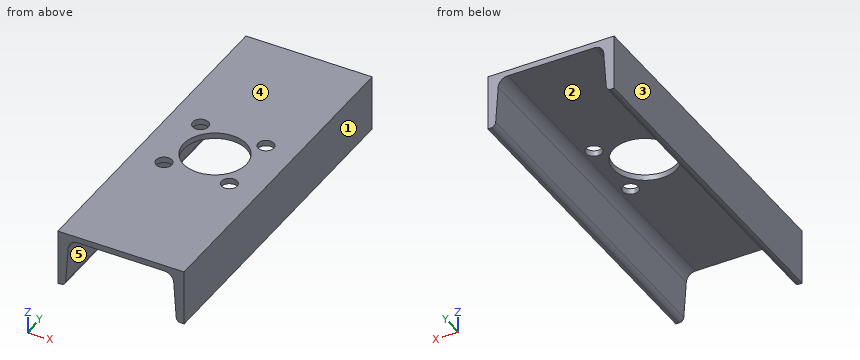
from build123d import *

# Parameters (mm, degrees)
MEMBER_12_1_DEPTH   = 320
SKETCH_5_R          = 30
SKETCH_5_R_2        = 7.5
CUT_EXTRUDE_1_DEPTH = 10


with BuildPart() as part:
    # Sketch1 → Member 12_1 (new body)
    with BuildSketch(Plane.ZX):
        with BuildLine():
            Line((0, 0), (0, -120))
            Line((0, -120), (-53, -120))
            Line((-53, -120), (-53, -117.0157841))
            ThreePointArc((-53, -117.0157841), (-51.788791155, -113.944326346), (-48.807176562, -112.526280502))
            Line((-48.807176562, -112.526280502), (-13.885646876, -110.136912681))
            ThreePointArc((-13.885646876, -110.136912681), (-7.922417689, -107.300820993), (-5.5, -101.157905484))
            Line((-5.5, -101.157905484), (-5.5, -18.842094516))
            ThreePointArc((-5.5, -18.842094516), (-7.922417689, -12.699179007), (-13.885646876, -9.863087319))
            Line((-13.885646876, -9.863087319), (-48.807176562, -7.473719498))
            ThreePointArc((-48.807176562, -7.473719498), (-51.788791155, -6.055673654), (-53, -2.9842159))
            Line((-53, -2.9842159), (-53, 0))
            Line((-53, 0), (0, 0))
        make_face()
    extrude(amount=MEMBER_12_1_DEPTH)

    # 草图5 → 切除-拉伸1 (cut)
    with BuildSketch(Plane.XY):
        with Locations((-60, 160)):
            Circle(SKETCH_5_R)
        with Locations((-91.112698372, 191.112698372)):
            Circle(SKETCH_5_R_2)
        with Locations((-28.887301628, 191.112698372)):
            Circle(SKETCH_5_R_2)
        with Locations((-28.887301628, 128.887301628)):
            Circle(SKETCH_5_R_2)
        with Locations((-91.112698372, 128.887301628)):
            Circle(SKETCH_5_R_2)
    extrude(amount=-CUT_EXTRUDE_1_DEPTH, mode=Mode.SUBTRACT)


solid = part.part
Read the model definition and answer for the solid it produces. Units are mm, in the model's axes. Face numbers are marked on the shaded views. A direction names the side the tool comes from. Round coordinates to 2 decimals unless told otherwise and drop trailing zeros. Write each loop counter-clockwise with the first axis right and the second up, starting at its lowest first coordinate (ties: lowest second). Pieces come first, ordered by that corner, then holes. Notation, with made-up numbers: (-36.75, 7) - (-3.75, 7) arc R12 ccw to (-3.75, 13) - close; hole circle Ø6 at (20.25, -3). An arc over 180 degrees is marked (long way). Use a Markdown table: item, result.
(1) The mould has two halves that part along X. Classify the marked faces 3, 4 and 5: released by +X, released by -X, zero draft, split by the parting line, or undercut.
Reported:
| item | result |
|---|---|
| face 3 | released by -X |
| face 4 | zero draft |
| face 5 | undercut |
(2) Each of these flat-tipped pins is pushed along its axis until it touches: pin 1 Ø17 at (x, y) = (-91.11, 128.89) entering from +Z; pin 2 Ø5 at (x, y) = (-30, 147.5) entering from -Z; pin 3 Ø9 at (x, y) = (-28.89, 191.11) entering from -Z. Where does it stop, or does it pass through?
Reported:
| item | result |
|---|---|
| pin 1 | z = 0 |
| pin 2 | z = -5.5 |
| pin 3 | through |
(3) The part is cut by section C-C (z = -23). Write down the section's boundary in (x, y), then the cut area to 3 significant figures.
Reported:
| item | result |
|---|---|
| outline | (-120, 0) - (-110.76, 0) - (-110.76, 320) - (-120, 320) - close; (-9.24, 0) - (0, 0) - (0, 320) - (-9.24, 320) - close |
| area | 5,910 mm2 |
(4) Straight lines are drawn through the part: line 1 along X through (y, z) = (29, -49); line 2 along Z through (x, y) = (-20.5, 15.5); line 3 along X through (y, z) = (273, -29.5). For each, find the intervals that lie inside material, in ascending order. Write a range as [from, to].
Reported:
| item | result |
|---|---|
| line 1 | [-120, -112.54], [-7.46, 0] |
| line 2 | [-5.5, 0] |
| line 3 | [-120, -111.21], [-8.79, 0] |
(5) The part is cut by section D-D (y = 271). Write down the section's boundary in (x, z).
Reported:
| item | result |
|---|---|
| outline | (-120, -53) - (-117.02, -53) arc R4.5 ccw to (-112.53, -48.81) - (-110.14, -13.89) arc R9 cw to (-101.16, -5.5) - (-18.84, -5.5) arc R9 cw to (-9.86, -13.89) - (-7.47, -48.81) arc R4.5 ccw to (-2.98, -53) - (0, -53) - (0, 0) - (-120, 0) - close |
(6) The part is cut by section A-A (y = 160). Write down the section's boundary in (x, z), then the cut area to 3 significant figures.
Reported:
| item | result |
|---|---|
| outline | (-120, -53) - (-117.02, -53) arc R4.5 ccw to (-112.53, -48.81) - (-110.14, -13.89) arc R9 cw to (-101.16, -5.5) - (-90, -5.5) - (-90, 0) - (-120, 0) - close; (-30, -5.5) - (-18.84, -5.5) arc R9 cw to (-9.86, -13.89) - (-7.47, -48.81) arc R4.5 ccw to (-2.98, -53) - (0, -53) - (0, 0) - (-30, 0) - close |
| area | 1,190 mm2 |
(7) Which of the six approach directions +Z, -Z, +X, -X, +Y, -Y give full straight-line access (tool end or side, diameter ignored) to the marked faces 1 and 2?
Reported:
| item | result |
|---|---|
| face 1 | +Z, -Z, +X, +Y, -Y |
| face 2 | -Z, +Y, -Y |
(8) The part is cut by section B-B (x = -60). Write down the section's boundary in (y, z), then the cut area to 3 significant figures.
Reported:
| item | result |
|---|---|
| outline | (0, -5.5) - (130, -5.5) - (130, 0) - (0, 0) - close; (190, -5.5) - (320, -5.5) - (320, 0) - (190, 0) - close |
| area | 1,430 mm2 |
